The listing builds one solid part. Answer for the finished solid, in the listing's coordinates (mm). Give positions to 0.01 mm unless a question says otherwise; leave off trailing zeros. Order: outer loops, then holes, each group sorted by start corner. A loop starts at its lowest first (then second) coordinate and runs counter-clockwise, first axis right, second up. Notation, with made-up numbers: (79, -35.75) - (105, -35.75) arc R26 cw to (105, -20.75) - close; hole circle Ø2 at (-24.5, 12). An arc over 180 degrees is marked (long way). Answer in a Markdown table with one row per item.
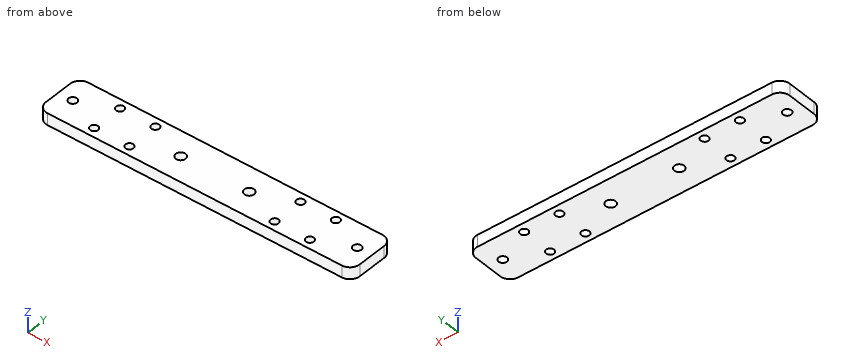
from build123d import *

# Parameters (mm, degrees)
SKETCH1_W              = 320
SKETCH1_H              = 50
SKETCH1_R              = 4
SKETCH1_R_2            = 5
BOSS_EXTRUDE1_DEPTH    = 12
M10_TAPPED_HOLE1_D     = 8.5
M10_TAPPED_HOLE1_DEPTH = 24.5
M10_TAPPED_HOLE1_TIP   = 2.553657631
FILLET1_R              = 10


with BuildPart() as part:
    # Sketch1 → Boss-Extrude1 (new body)
    with BuildSketch(Plane.XY):
        with Locations((160, 25)):
            Rectangle(SKETCH1_W, SKETCH1_H)
        with Locations((50, 41)):
            Circle(SKETCH1_R, mode=Mode.SUBTRACT)
        with Locations((86, 41)):
            Circle(SKETCH1_R, mode=Mode.SUBTRACT)
        with Locations(Location((86, 9, 0), (0, 0, 180))):
            Circle(SKETCH1_R, mode=Mode.SUBTRACT)
        with Locations(Location((50, 9, 0), (0, 0, 180))):
            Circle(SKETCH1_R, mode=Mode.SUBTRACT)
        with Locations((270, 9)):
            Circle(SKETCH1_R, mode=Mode.SUBTRACT)
        with Locations((234, 9)):
            Circle(SKETCH1_R, mode=Mode.SUBTRACT)
        with Locations(Location((234, 41, 0), (0, 0, 180))):
            Circle(SKETCH1_R, mode=Mode.SUBTRACT)
        with Locations(Location((270, 41, 0), (0, 0, 180))):
            Circle(SKETCH1_R, mode=Mode.SUBTRACT)
        with Locations((125, 25)):
            Circle(SKETCH1_R_2, mode=Mode.SUBTRACT)
        with Locations((195, 25)):
            Circle(SKETCH1_R_2, mode=Mode.SUBTRACT)
    extrude(amount=BOSS_EXTRUDE1_DEPTH)

    # M10 Tapped Hole1
    with Locations(Plane.XY.offset(12)):
        with Locations((15, 25), (305, 25)):
            Hole(M10_TAPPED_HOLE1_D / 2, depth=M10_TAPPED_HOLE1_DEPTH)
            with Locations((0, 0, -(M10_TAPPED_HOLE1_DEPTH + M10_TAPPED_HOLE1_TIP / 2))):  # 118° drill point
                Cone(0, M10_TAPPED_HOLE1_D / 2, M10_TAPPED_HOLE1_TIP, mode=Mode.SUBTRACT)

    # Fillet1
    fillet1_edges = [part.edges().sort_by_distance(p)[0] for p in [
        (320, 0, 6),
        (0, 0, 6),
        (0, 50, 6),
        (320, 50, 6),
    ]]
    fillet(fillet1_edges, radius=FILLET1_R)


solid = part.part
Item 1: Find section C-C on y = 25. Write down the section's boundary in (x, z).
Answer block:
| item | result |
|---|---|
| outline | (0, 0) - (10.75, 0) - (10.75, 12) - (0, 12) - close; (19.25, 0) - (120, 0) - (120, 12) - (19.25, 12) - close; (130, 0) - (190, 0) - (190, 12) - (130, 12) - close; (200, 0) - (300.75, 0) - (300.75, 12) - (200, 12) - close; (309.25, 0) - (320, 0) - (320, 12) - (309.25, 12) - close |
Item 2: Consider line 1 (Y direction, x = 234, z = 5.5); line 2 (X direction, y = 21.5, z = 3); line 3 (X direction, y = 29.5, z = 2.75). Determine where each line is inside the solid, lowest interval first.
Answer block:
| item | result |
|---|---|
| line 1 | 0 to 5, 13 to 37, 45 to 50 |
| line 2 | 0 to 12.59, 17.41 to 121.43, 128.57 to 191.43, 198.57 to 302.59, 307.41 to 320 |
| line 3 | 0 to 122.82, 127.18 to 192.82, 197.18 to 320 |
Item 3: Find section A-A on x = 15. Write down the section's boundary in (y, z), then the cut area to 3 significant figures.
Answer block:
| item | result |
|---|---|
| outline | (0, 0) - (20.75, 0) - (20.75, 12) - (0, 12) - close; (29.25, 0) - (50, 0) - (50, 12) - (29.25, 12) - close |
| area | 498 mm² |
Item 4: Find section B-B on z = 9. Count the separate pieces of the cut face and the enclosed holes in it, then the cut area to 3 significant figures.
Answer block:
| item | result |
|---|---|
| separate pieces | 1 |
| enclosed holes | 12 |
| area | 15,200 mm² |
Item 5: This flat-tipped pin is pushed along its axis until it touches: P1, Ø2, axis at y = 9, z = 9, coming from the -X side. Where does it stop, or does it pass through?
Answer block:
| item | result |
|---|---|
| P1 | x = 0 |
Item 6: Find section D-D on x = 234. Write down the section's boundary in (y, z).
Answer block:
| item | result |
|---|---|
| outline | (0, 0) - (5, 0) - (5, 12) - (0, 12) - close; (13, 0) - (37, 0) - (37, 12) - (13, 12) - close; (45, 0) - (50, 0) - (50, 12) - (45, 12) - close |
